from build123d import *

# Parameters (mm, degrees)
SKETCH2_R = 6


with BuildPart() as part:
    # Sweep1: sweep along a path in Sketch1
    with BuildLine(Plane.XY) as sweep1_path:
        Line((-49.237651445, -16.859273066), (-49.237651445, 26.640726934))
        ThreePointArc((-49.237651445, 26.640726934), (-47.333845522, 31.236921012), (-42.737651445, 33.140726934))
        Line((-42.737651445, 33.140726934), (763.262348555, 33.140726934))
        ThreePointArc((763.262348555, 33.140726934), (767.858542633, 31.236921012), (769.762348555, 26.640726934))
        Line((769.762348555, 26.640726934), (769.762348555, -16.859273066))
    # Sketch2 → Sweep1 (sweep)
    with BuildSketch(Plane(origin=(-49.237651445, -16.859273066, 0), x_dir=(-1, 0, 0), z_dir=(0, 1, 0))):
        Circle(SKETCH2_R)
    sweep(path=sweep1_path.line)


solid = part.part
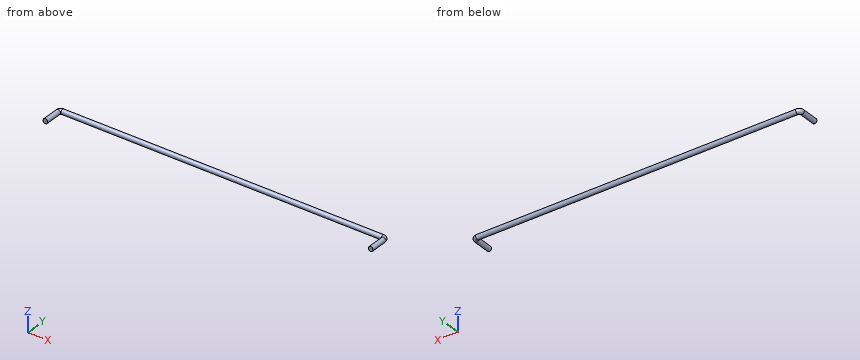
Check sheet for the modelled part. Datum: model origin and axes. Units: mm. Coordinates: 2 decimals unless noted, no trailing zeros. Write each loop counter-clockwise with the first axis right and the second up, starting at its lowest first coordinate (ties: lowest second). Pieces come first, ordered by that corner, then holes.
Item 1: Cross-section at A-A on y = 11. Record the boundary of the cut face in (x, z), then the cut area to 3 significant figures.
Numbers:
outline: circle Ø12 at (-49.24, 0); circle Ø12 at (769.76, 0)
area: 226 mm2
Item 2: Depth check by flat-ended pin: pin 1 Ø3 at (x, z) = (617.5, -0.5) entering from -Y; pin 2 Ø1 at (y, z) = (-4.5, 3) entering from -X; pin 3 Ø4 at (x, z) = (464.5, -4) entering from -Y. Enter the tip coordinate at first touch or a pass-through.
Numbers:
pin 1: stops at y = 27.14
pin 2: stops at x = -54.69
pin 3: stops at y = 27.48
Item 3: Scan lines: probe 1 along X at (y, z) = (17.5, -1); probe 2 along Y at (x, z) = (308, 1.25); probe 3 along X at (y, z) = (22, -0.25). Record each from-to range of solid material in increasing order.
Numbers:
probe 1: x = -55.15 to -43.32, 763.85 to 775.68
probe 2: y = 27.27 to 39.01
probe 3: x = -55.23 to -43.24, 763.77 to 775.76
